from build123d import *

# Parameters (mm, degrees)
EXTRUDE_1_DEPTH = 34


with BuildPart() as part:
    # 草图1 → 拉伸-薄壁1 (new, symmetric)
    with BuildSketch(Plane(origin=(-86.992315928, -141.229957863, -135.692636998), x_dir=(0, 0, -1), z_dir=(-1, 0, 0))):
        with BuildLine():
            Line((1100, 0), (-695.31480211, 0))
            ThreePointArc((-695.31480211, 0), (-761.535134985, 66.220332876), (-695.31480211, 132.440665751))
            Line((-695.31480211, 132.440665751), (-203.750159412, 132.440665751))
            Line((-203.750159412, 132.440665751), (-203.750159412, 97.440665751))
            Line((-203.750159412, 97.440665751), (-695.31480211, 97.440665751))
            ThreePointArc((-695.31480211, 97.440665751), (-726.535134985, 66.220332876), (-695.31480211, 35))
            Line((-695.31480211, 35), (1100, 35))
            Line((1100, 35), (1100, 0))
        make_face()
    extrude(amount=EXTRUDE_1_DEPTH, both=True)


solid = part.part
The listing builds one solid part. Answer for the finished solid, in the listing's coordinates (mm). A direction names the side the tool comes from. Coordinates: 2 decimals unless noted, no trailing zeros. Loops run counter-clockwise (first coordinate to the right, second up) from the corner with the lowest first, then second, coordinate; pieces in that order, holes last. Notation, with made-up numbers: (30.5, 44) -> (81.5, 44) arc R19 cw to (81.5, 53) -> close; hole circle Ø10 at (-19.5, -6). An arc over 180 degrees is marked (long way). Write item = value, one per line. Start each with the question number.
1) A cutting plane is placed at A-A (z = 411). Give the vertices of the cut face in (x, y), then the cut area to 3 significant figures.
2) Given pin 1 Ø10 at (x, y) = (-102, -239) entering from +Z; pin 2 Ø6 at (x, y) = (-88.5, -232.5) entering from -Z; pin 3 Ø10 at (x, z) = (-82, -168.5) entering from -Y, each flat-ended and moving along its own axis, determine where each tip first touches the part or whether it passes through.
3) The mould has two halves that part along Y. Classify faces 1 (the face through (-87, -238.671, 310)), 2 (the face through (-52.992, -173, -171)), 3 (the face through (-87, -141.23, -351)): released by +Y, released by -Y, zero draft, split by the parting line, or undercut.
4) Straight lines are drawn through the part: line 1 (Y direction, x = -65.5, z = 415); line 2 (Y direction, x = -103, z = -510.5); line 3 (Z direction, x = -105, y = -227.5). For each, find the intervals that lie inside material, in ascending order. Write a range as from..to.
5) A tool of negligible diameter and unlimited length cuts with its end or side. For faces 4 (the face through (-87, -256, 68.058)), 5 (the face through (-87, -273.671, 317)), 6 (the face through (-87, -176.23, -325)), from which of +Z, -Z, +X, -X, +Y, -Y can it reach the whole face along a straight path? Write none if from no direction.
6) A cutting plane is placed at B-B (x = -65.5). Give the vertices of the cut face in (y, z).
7) A cutting plane is placed at C-C (z = -625). Give the vertices of the cut face in (x, y).
Responses:
q1.outline = (-120.99, -273.67) -> (-52.99, -273.67) -> (-52.99, -238.67) -> (-120.99, -238.67) -> close; (-120.99, -176.23) -> (-52.99, -176.23) -> (-52.99, -141.23) -> (-120.99, -141.23) -> close
q1.area = 4,760 mm²
q2.pin_1 = 620.29
q2.pin_2 = 573.33
q2.pin_3 = -176.23
q3.face_1 = undercut
q3.face_2 = zero draft
q3.face_3 = released by +Y
q4.line_1 = -273.67..-238.67, -176.23..-141.23
q4.line_2 = -176.23..-141.23
q4.line_3 = 583.55..622.73
q5.face_4 = -Z, +X, -X, -Y
q5.face_5 = +Z, -Z, +X, -X, -Y
q5.face_6 = -Z, +X, -X
q6.outline = (-273.67, 68.06) -> (-238.67, 68.06) -> (-238.67, 559.62) arc R31.22 cw to (-176.23, 559.62) -> (-176.23, -1235.69) -> (-141.23, -1235.69) -> (-141.23, 559.62) arc R66.22 ccw to (-273.67, 559.62) -> close
q7.outline = (-120.99, -176.23) -> (-52.99, -176.23) -> (-52.99, -141.23) -> (-120.99, -141.23) -> close
